```python
from build123d import *

# Parameters (mm, degrees)
SKETCH1_R           = 5
BOSS_EXTRUDE1_DEPTH = 400


with BuildPart() as part:
    # Sketch1 → Boss-Extrude1 (new body)
    with BuildSketch(Plane(origin=(0, 0, 0), x_dir=(1, 0, 0), z_dir=(0, 1, 0))):
        Polygon((-6, 20), (-6, 16), (-11.757359313, 16), (-5.757359313, 10), (5.757359313, 10), (11.757359313, 16), (6, 16), (6, 20), (20, 20), (20, 6), (16, 6), (16, 11.757359313), (10, 5.757359313), (10, -5.757359313), (16, -11.757359313), (16, -6), (20, -6), (20, -20), (6, -20), (6, -16), (11.757359313, -16), (5.757359313, -10), (-5.757359313, -10), (-11.757359313, -16), (-6, -16), (-6, -20), (-20, -20), (-20, -6), (-16, -6), (-16, -11.757359313), (-10, -5.757359313), (-10, 5.757359313), (-16, 11.757359313), (-16, 6), (-20, 6), (-20, 20), align=None)
        with Locations(Location((0, 0, 0), (0, 0, 270))):
            Circle(SKETCH1_R, mode=Mode.SUBTRACT)
    extrude(amount=BOSS_EXTRUDE1_DEPTH)


solid = part.part
```
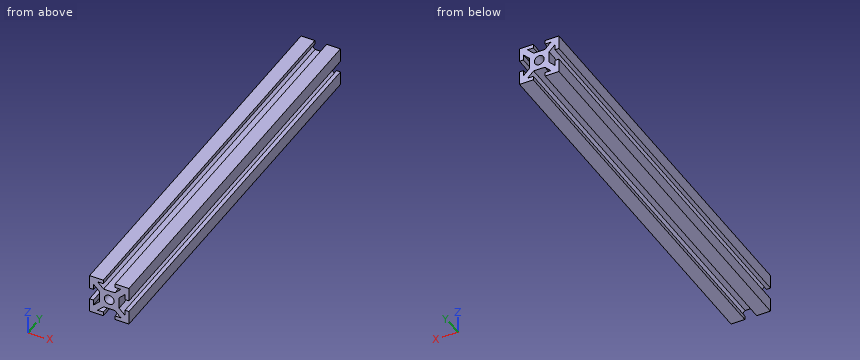
Source: CAD feature listing. Evaluate the final solid. Frame: model axes, mm. Give positions to 0.01 mm unless a question says otherwise; leave off trailing zeros. Write each loop counter-clockwise with the first axis right and the second up, starting at its lowest first coordinate (ties: lowest second). Pieces come first, ordered by that corner, then holes.
1. Section query A-A (x = 0). Return the cut outline in (y, z), then the cut area to 3 significant figures.
2. Material intervals for line 1 along Z through (x, y) = (17, 175.5); line 2 along X through (y, z) = (132.5, 6.5); line 3 along X through (y, z) = (166, 0), sorted ascending.
3. First-contact query: pin 1 (3.5 mm diameter, centred on y = 235, z = 2.5, fed in from +X); pin 2 (12.5 mm diameter, centred on x = -1, y = 128.5, fed in from -Z); pin 3 (8 mm diameter, centred on x = 0, z = 0, fed in from -Y). Flat tips, straight axial feed; report the tip coordinate or a pass-through.
4. Section query B-B (z = 0). Return the cut outline in (x, y).
Output values:
1. outline: (0, -10) - (400, -10) - (400, -5) - (0, -5) - close; (0, 5) - (400, 5) - (400, 10) - (0, 10) - close
1. area: 4,000 mm2
2. line 1: z = -20 to -6, 6 to 20
2. line 2: x = -20 to -16, -10.74 to 10.74, 16 to 20
2. line 3: x = -10 to -5, 5 to 10
3. pin 1: stops at x = 10
3. pin 2: stops at z = -20
3. pin 3: passes through
4. outline: (-10, 0) - (-5, 0) - (-5, 400) - (-10, 400) - close; (5, 0) - (10, 0) - (10, 400) - (5, 400) - close
